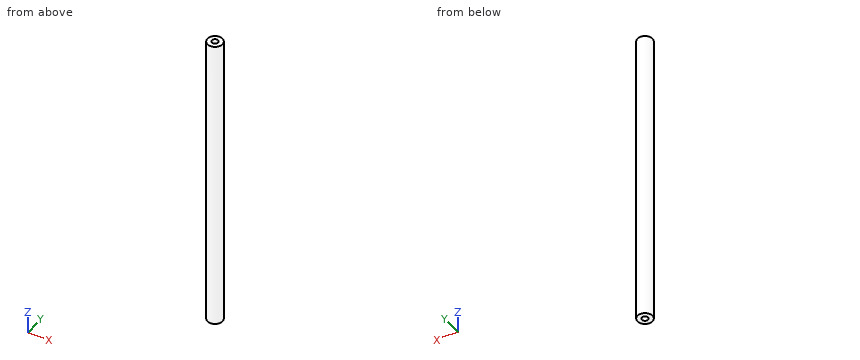
from build123d import *

# Parameters (mm, degrees)
SKETCH1_R             = 3
BOSS_EXTRUDE1_DEPTH   = 120
M3_TAPPED_HOLE1_D     = 2.5
M3_TAPPED_HOLE1_DEPTH = 8.5
M3_TAPPED_HOLE1_TIP   = 0.751075774
M3_TAPPED_HOLE2_D     = 2.5
M3_TAPPED_HOLE2_DEPTH = 8.5
M3_TAPPED_HOLE2_TIP   = 0.751075774


with BuildPart() as part:
    # Sketch1 → Boss-Extrude1 (new body)
    with BuildSketch(Plane.XY):
        Circle(SKETCH1_R)
    extrude(amount=BOSS_EXTRUDE1_DEPTH)

    # M3 Tapped Hole1
    with Locations(Plane.XY.offset(120)):
        with Locations((0, 0)):
            Hole(M3_TAPPED_HOLE1_D / 2, depth=M3_TAPPED_HOLE1_DEPTH)
            with Locations((0, 0, -(M3_TAPPED_HOLE1_DEPTH + M3_TAPPED_HOLE1_TIP / 2))):  # 118° drill point
                Cone(0, M3_TAPPED_HOLE1_D / 2, M3_TAPPED_HOLE1_TIP, mode=Mode.SUBTRACT)

    # M3 Tapped Hole2
    with Locations(Plane(origin=(0, 0, 0), x_dir=(-1, 0, 0), z_dir=(0, 0, -1))):
        with Locations((0, 0)):
            Hole(M3_TAPPED_HOLE2_D / 2, depth=M3_TAPPED_HOLE2_DEPTH)
            with Locations((0, 0, -(M3_TAPPED_HOLE2_DEPTH + M3_TAPPED_HOLE2_TIP / 2))):  # 118° drill point
                Cone(0, M3_TAPPED_HOLE2_D / 2, M3_TAPPED_HOLE2_TIP, mode=Mode.SUBTRACT)


solid = part.part
Can you work these out from the model? Positions are in its coordinate system, mm. Round coordinates to 2 decimals unless told otherwise and drop trailing zeros. Write each loop counter-clockwise with the first axis right and the second up, starting at its lowest first coordinate (ties: lowest second). Pieces come first, ordered by that corner, then holes. Notation, with made-up numbers: (-11, -23) -> (24, -23) arc R11 cw to (24, -12) -> close; hole circle Ø6 at (86, -39). An arc over 180 degrees is marked (long way). One line per question, with ' | ' between items. Start each with the question number.
1) I'm going to push flat-ended pins straight in: P1, Ø1.5, axis at y = -2, z = 85, coming from the +X side; P2, Ø2, axis at x = 0, y = 0, coming from the -Z side; P3, Ø2, axis at x = -2.5, z = 60.5, coming from the +Y side. Where does each tip first touch, or does it pass through?
2) I need wall thicknesses on line 1 (X direction, y = -0.25, z = 14); line 2 (Y direction, x = 0, z = 116.5); line 3 (X direction, y = 2.15, z = 104). Which ranges of each line are inside material? Lowest first, please. Write a range as [from, to].
3) Suppose I cut it at A-A on z = 48. Write out the boundary of the cut face in (x, y), then the cut area to 3 significant figures.
Return value:
1) P1: stops at x = 2.73 | P2: stops at z = 8.65 | P3: stops at y = 2.6
2) line 1: x = [-2.99, 2.99] | line 2: y = [-3, -1.25], [1.25, 3] | line 3: x = [-2.09, 2.09]
3) outline: circle Ø6 at (0, 0) | area: 28.3 mm2
